Study the drawing (mm; zero at the part's minimum x, y, z) and answer. Give positions to 0.01 mm unless a question says otherwise; leave off trailing zeros. Loops run counter-clockwise (first coordinate to the right, second up) from the corner with the lowest first, then second, coordinate; pieces in that order, holes last. Notation, with made-up numbers: (74.5, 70) - (82.5, 70) arc R17 cw to (82.5, 100) - close; hole circle Ø9 at (26.25, 48). An arc over 180 degrees is marked (long way). Answer in a Markdown table with one row per item. Add a question column.
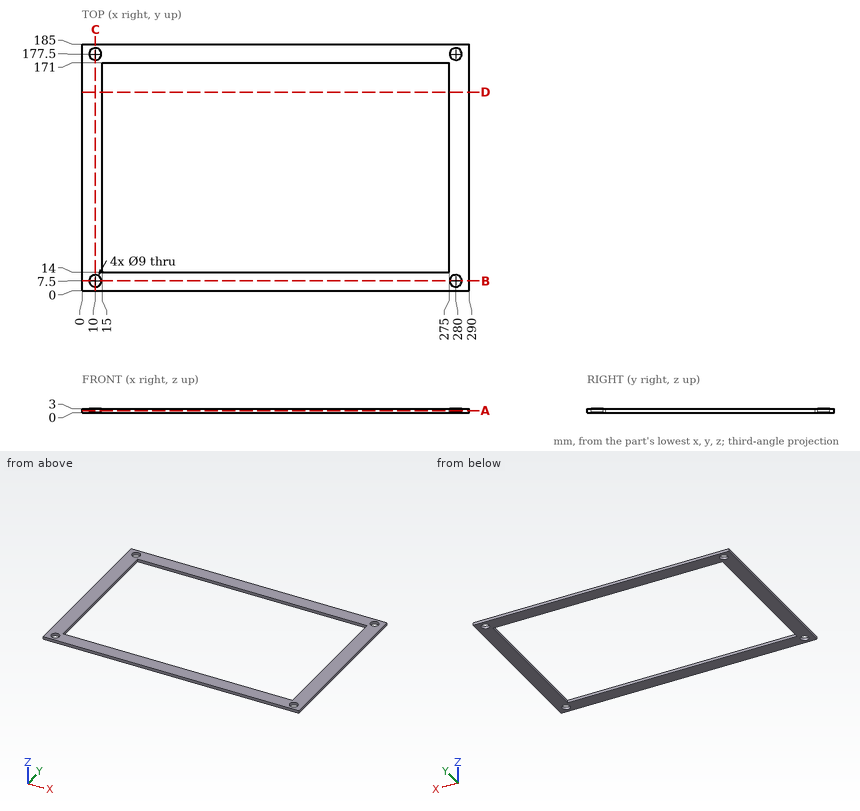
(1) Find the intervals of material crossed by line 1 along Y through (x, z) = (280, 2.1); line 2 along X through (y, z) = (177.5, 0.8); line 3 along Y through (x, z) = (53.5, 2.25), in increasing order. Write a range as [from, to].
(2) A cutting plane is placed at D-D on y = 149. Determine the outline of the cut face in (x, z), plus the area to 3 significant figures.
(3) A cutting plane is placed at A-A on z = 1.8. Determine the outline of the cut face in (x, y), plus the area to 3 significant figures.
(4) A cutting plane is placed at B-B on y = 7.5. Determine the outline of the cut face in (x, z), plus the area to 3 significant figures.
(5) A cutting plane is placed at C-C on x = 10. Determine the outline of the cut face in (y, z), plus the area to 3 significant figures.
Evaluation:
| question | item | result |
|---|---|---|
| 1 | line 1 | y = [0, 3], [12, 173], [182, 185] |
| 1 | line 2 | x = [0, 5.5], [14.5, 275.5], [284.5, 290] |
| 1 | line 3 | y = [0, 14], [171, 185] |
| 2 | outline | (0, 0) - (15, 0) - (15, 3) - (0, 3) - close; (275, 0) - (290, 0) - (290, 3) - (275, 3) - close |
| 2 | area | 90.0 mm² |
| 3 | outline | (0, 0) - (290, 0) - (290, 185) - (0, 185) - close; hole circle Ø9 at (10, 7.5); hole circle Ø9 at (10, 177.5); hole (15, 14) - (275, 14) - (275, 171) - (15, 171) - close; hole circle Ø9 at (280, 7.5); hole circle Ø9 at (280, 177.5) |
| 3 | area | 12,600 mm² |
| 4 | outline | (0, 0) - (5.5, 0) - (5.5, 3) - (0, 3) - close; (14.5, 0) - (275.5, 0) - (275.5, 3) - (14.5, 3) - close; (284.5, 0) - (290, 0) - (290, 3) - (284.5, 3) - close |
| 4 | area | 816 mm² |
| 5 | outline | (0, 0) - (3, 0) - (3, 3) - (0, 3) - close; (12, 0) - (173, 0) - (173, 3) - (12, 3) - close; (182, 0) - (185, 0) - (185, 3) - (182, 3) - close |
| 5 | area | 501 mm² |
